```python
from build123d import *

# Parameters (mm, degrees)
SKETCH1_R           = 3
SKETCH1_R_2         = 2
BOSS_EXTRUDE1_DEPTH = 5


with BuildPart() as part:
    # Sketch1 → Boss-Extrude1 (new body)
    with BuildSketch(Plane.XY):
        with BuildLine():
            Line((-7.5, 0), (-7.5, 17.073921172))
            ThreePointArc((-7.5, 17.073921172), (-7.247513667, 18.278565788), (-6.532554233, 19.280439536))
            Line((-6.532554233, 19.280439536), (6.669927689, 31.442024485))
            ThreePointArc((6.669927689, 31.442024485), (12.26799775, 31.26757457), (12.204, 25.667152669))
            ThreePointArc((12.204, 25.667152669), (8.722720142, 20.47025599), (7.5, 14.335763346))
            Line((7.5, 14.335763346), (7.5, 0))
            ThreePointArc((7.5, 0), (0, -7.5), (-7.5, 0))
        make_face()
        Circle(SKETCH1_R, mode=Mode.SUBTRACT)
        with Locations((2.5, 19.5)):
            Circle(SKETCH1_R_2, mode=Mode.SUBTRACT)
        with Locations((9.38, 28.5)):
            Circle(SKETCH1_R_2, mode=Mode.SUBTRACT)
    extrude(amount=BOSS_EXTRUDE1_DEPTH)


solid = part.part
```
Here's how the part is built. I have some questions about the finished solid (model axes, mm). A direction names the side the tool comes from. Round coordinates to 2 decimals unless told otherwise and drop trailing zeros. Order: outer loops, then holes, each group sorted by start corner. A loop starts at its lowest first (then second) coordinate and runs counter-clockwise, first axis right, second up. Notation, with made-up numbers: (-6.75, -26.75) -> (12.25, -26.75) arc R35 cw to (12.25, 6.25) -> close; hole circle Ø8 at (11, -38.75). An arc over 180 degrees is marked (long way). Use a Markdown table: item, result. Add a question column.
(1) Suppose I cut it at C-C, the plane z = 4.2. Please give me the cut outline in (x, y).
(2) Suppose I cut it at D-D, the plane y = 11. Please give me the cut outline in (x, z).
(3) For faces 1 (the face through (7.5, 7, 2)), 2 (the face through (-7.254, 18.263, 2.465)), which set-ups out of +Z, -Z, +X, -X, +Y, -Y let a thin tool reach every point of the face, with its end or its side?
(4) If we mould it in two halves opening along Y, with no side actions, what happens to faces 3 (the face through (10.303, 26.726, 2.465)), 4 (the face through (0.16, -7.5, 2.46)), 5 (the face through (-7.5, 8, 2))? For each: released by +Y, released by -Y, zero draft, split by the parting line, or undercut.
(5) Suppose I cut it at A-A, the plane x = 9.38. Please give me the cut outline in (y, z).
(6) For pin 1 Ø2.5 at (x, y) = (2.5, 19.5) entering from +Z; pin 2 Ø2 at (x, z) = (4, 3.5) entering from -Y; pin 3 Ø3 at (y, z) = (16.5, 0.5) entering from +X; pin 4 Ø3 at (x, z) = (-5, 2.5) entering from -Y, each with a flat end and sliding along its axis, tell me the tip position at first contact or that it passes through.
(7) Suppose I cut it at B-B, the plane y = 28.5. Please give me the cut outline in (x, z), and give its area (3 significant figures).
(8) I need wall thicknesses on line 1 along Y through (x, z) = (2.5, 2.45); line 2 along Y through (x, z) = (2.25, 4.2); line 3 along X through (y, z) = (7.5, 3.95). Which ranges of each line are inside material? Lowest first, please.
Verdict:
| question | item | result |
|---|---|---|
| 1 | outline | (-7.5, 0) arc R7.5 ccw to (7.5, 0) -> (7.5, 14.34) arc R16 cw to (12.2, 25.67) arc R4 ccw to (6.67, 31.44) -> (-6.53, 19.28) arc R3 ccw to (-7.5, 17.07) -> close; hole circle Ø6 at (0, 0); hole circle Ø4 at (2.5, 19.5); hole circle Ø4 at (9.38, 28.5) |
| 2 | outline | (-7.5, 0) -> (7.5, 0) -> (7.5, 5) -> (-7.5, 5) -> close |
| 3 | face 1 | +Z, -Z, +X, -Y |
| 3 | face 2 | +Z, -Z, -X, +Y |
| 4 | face 3 | undercut |
| 4 | face 4 | released by -Y |
| 4 | face 5 | zero draft |
| 5 | outline | (21.86, 0) -> (26.5, 0) -> (26.5, 5) -> (21.86, 5) -> close; (30.5, 0) -> (32.5, 0) -> (32.5, 5) -> (30.5, 5) -> close |
| 6 | pin 1 | through |
| 6 | pin 2 | y = -6.87 |
| 6 | pin 3 | x = 7.93 |
| 6 | pin 4 | y = -6.63 |
| 7 | outline | (3.48, 0) -> (7.38, 0) -> (7.38, 5) -> (3.48, 5) -> close; (11.38, 0) -> (13.38, 0) -> (13.38, 5) -> (11.38, 5) -> close |
| 7 | area | 29.5 mm2 |
| 8 | line 1 | -7.07 to -1.66, 1.66 to 17.5, 21.5 to 27.6 |
| 8 | line 2 | -7.15 to -1.98, 1.98 to 17.52, 21.48 to 27.37 |
| 8 | line 3 | -7.5 to 7.5 |
